CAD build for the part. Positions are in the model's coordinates, mm. Coordinates: 2 decimals unless noted, no trailing zeros. Loops run counter-clockwise (first coordinate to the right, second up) from the corner with the lowest first, then second, coordinate; pieces in that order, holes last. Notation, with made-up numbers: (25.5, 2) -> (42.5, 2) arc R20 cw to (42.5, 41) -> close; hole circle Ø3 at (19.25, 33.25). An arc over 180 degrees is marked (long way). Write each question's results on one line, items separated by ' | '.
from build123d import *

# Parameters (mm, degrees)
SKETCH_1_W             = 830
SKETCH_1_H             = 2008
SKETCH_1_W_2           = 620
SKETCH_1_H_2           = 850
EXTRUDE_1_DEPTH        = 2
SKETCH_2_W             = 810
SKETCH_2_H             = 30
CUT_EXTRUDE_1_DEPTH    = 2
SKETCH_3_W             = 2
SKETCH_3_H             = 2008
EXTRUDE_2_DEPTH        = 25.5
SKETCH_4_W             = 200
SKETCH_4_H             = 150
CUT_EXTRUDE_2_DEPTH    = 2173.927575875
SKETCH_5_W             = 30
SKETCH_5_H             = 2
SKETCH_5_W_2           = 596
SKETCH_5_W_3           = 826
EXTRUDE_3_DEPTH        = 25.5
EXTRUDE_4_DEPTH        = 5
SKETCH_8_W             = 3
SKETCH_8_H             = 8
CUT_EXTRUDE_3_DEPTH    = 813
PATTERN_LINEAR_1_COUNT = 2
PATTERN_LINEAR_1_PITCH = 1050
SKETCH_9_R             = 2.75
CUT_EXTRUDE_4_DEPTH    = 126
SKETCH_10_R            = 2.75
CUT_EXTRUDE_5_DEPTH    = 1163


with BuildPart() as part:
    # 草图1 → 凸台-拉伸1 (new body)
    with BuildSketch(Plane.XY):
        with Locations((415, -1004)):
            Rectangle(SKETCH_1_W, SKETCH_1_H)
        with Locations((415, -1133)):
            Rectangle(SKETCH_1_W_2, SKETCH_1_H_2, mode=Mode.SUBTRACT)
    extrude(amount=EXTRUDE_1_DEPTH)

    # 草图2 → 切除-拉伸1 (cut)
    with BuildSketch(Plane.XY.offset(2)):
        with Locations((415, -1658)):
            Rectangle(SKETCH_2_W, SKETCH_2_H)
        with Locations((415, -608)):
            Rectangle(SKETCH_2_W, SKETCH_2_H)
    extrude(amount=-CUT_EXTRUDE_1_DEPTH, mode=Mode.SUBTRACT)

    # 草图3 → 凸台-拉伸2 (add)
    with BuildSketch(Plane.XY):
        with Locations((1, -1004)):
            Rectangle(SKETCH_3_W, SKETCH_3_H)
        with Locations((829, -1004)):
            Rectangle(SKETCH_3_W, SKETCH_3_H)
    extrude(amount=-EXTRUDE_2_DEPTH)

    # 草图4 → 切除-拉伸2 (cut, through all)
    with BuildSketch(Plane(origin=(0, 0, 0), x_dir=(-1, 0, 0), z_dir=(0, 0, -1))):
        with Locations((-698, -1933)):
            Rectangle(SKETCH_4_W, SKETCH_4_H)
    extrude(amount=-CUT_EXTRUDE_2_DEPTH, mode=Mode.SUBTRACT)

    # 草图5 → 凸台-拉伸3 (add)
    with BuildSketch(Plane(origin=(0, 0, 0), x_dir=(-1, 0, 0), z_dir=(0, 0, -1))):
        with Locations((-813, -2007)):
            Rectangle(SKETCH_5_W, SKETCH_5_H)
        with Locations((-300, -2007)):
            Rectangle(SKETCH_5_W_2, SKETCH_5_H)
        with Locations((-415, -1)):
            Rectangle(SKETCH_5_W_3, SKETCH_5_H)
    extrude(amount=EXTRUDE_3_DEPTH)

    # 草图7 → 凸台-拉伸4 (add)
    with BuildSketch(Plane.XY.offset(2)):
        Polygon((820, -564.997302091), (820, -580), (7, -580), (7, -636), (820, -636), (820, -651), (0, -651), (0, -564.997302091), align=None)
    extrude_4 = extrude(amount=EXTRUDE_4_DEPTH)

    # 草图8 → 切除-拉伸3 (cut)
    with BuildSketch(Plane(origin=(820, 0, 0), x_dir=(0, 0, -1), z_dir=(1, 0, 0))):
        with Locations((-3.5, -576)):
            Rectangle(SKETCH_8_W, SKETCH_8_H)
        with Locations((-3.5, -640)):
            Rectangle(SKETCH_8_W, SKETCH_8_H)
    cut_extrude_3 = extrude(amount=-CUT_EXTRUDE_3_DEPTH, mode=Mode.SUBTRACT)

    # 阵列(线性)1: 凸台-拉伸4, 切除-拉伸3 ×2
    with Locations(*[(0, -i * PATTERN_LINEAR_1_PITCH, 0) for i in range(1, PATTERN_LINEAR_1_COUNT)]):
        add(extrude_4)
        add(cut_extrude_3, mode=Mode.SUBTRACT)

    # 草图9 → 切除-拉伸4 (cut)
    with BuildSketch(Plane(origin=(0, 0, 0), x_dir=(-1, 0, 0), z_dir=(0, 0, -1))):
        with Locations((-565, -695.5)):
            Circle(SKETCH_9_R)
        with Locations((-265, -695.5)):
            Circle(SKETCH_9_R)
        with Locations((-737.5, -933)):
            Circle(SKETCH_9_R)
        with Locations((-737.5, -1333)):
            Circle(SKETCH_9_R)
        with Locations((-565, -1570.5)):
            Circle(SKETCH_9_R)
        with Locations((-265, -1570.5)):
            Circle(SKETCH_9_R)
        with Locations((-92.5, -1333)):
            Circle(SKETCH_9_R)
        with Locations((-92.5, -933)):
            Circle(SKETCH_9_R)
    extrude(amount=-CUT_EXTRUDE_4_DEPTH, mode=Mode.SUBTRACT)

    # 草图10 → 切除-拉伸5 (cut)
    with BuildSketch(Plane.ZY):
        with Locations(Location((-16.5, -1978, 0), (0, 0, 270))):
            Circle(SKETCH_10_R)
        with Locations(Location((-16.5, -1158, 0), (0, 0, 270))):
            Circle(SKETCH_10_R)
        with Locations(Location((-16.5, -338, 0), (0, 0, 270))):
            Circle(SKETCH_10_R)
    extrude(amount=-CUT_EXTRUDE_5_DEPTH, mode=Mode.SUBTRACT)


solid = part.part
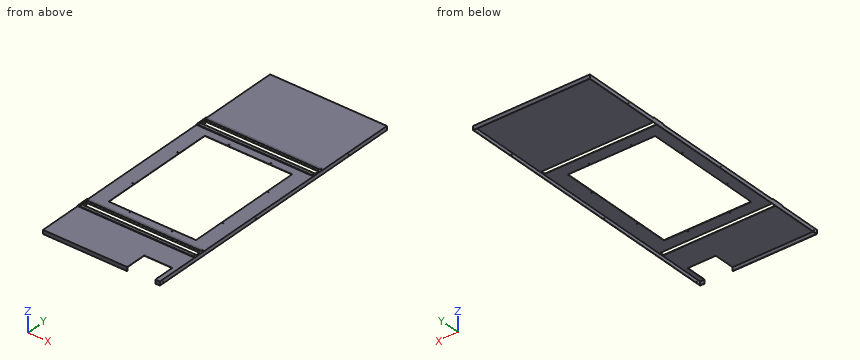
1) Slice it at B-B (x = 534). Count the separate pieces of the cut face and the enclosed holes in it, then the cut area to 3 significant figures.
Outcome:
separate pieces: 4 | enclosed holes: 0 | area: 2,500 mm^2
2) Drill centre lines: L1, parallel to X at y = -1570.5, z = 1.35; L2, parallel to Y at x = 737.5, z = 1.3; L3, parallel to X at y = -1333, z = 1. Where is each one in solid material? Low to high. Write a range as from..to.
Outcome:
L1: x = 0..262.25, 267.75..562.25, 567.75..830 | L2: y = -1858..-1673, -1643..-1335.75, -1330.25..-935.75, -930.25..-623, -593..0 | L3: x = 0..89.75, 95.25..105, 725..734.75, 740.25..830
3) Slice it at C-C (z = -6). Write the cut outline in (x, y), then the cut area to 3 significant figures.
Outcome:
outline: (0, -2008) -> (598, -2008) -> (598, -2006) -> (2, -2006) -> (2, -2) -> (828, -2) -> (828, -2006) -> (798, -2006) -> (798, -2008) -> (830, -2008) -> (830, 0) -> (0, 0) -> close | area: 10,900 mm^2
4) Slice it at D-D (y = -1083.5). Write the cut outline in (x, z).
Outcome:
outline: (0, -25.5) -> (2, -25.5) -> (2, 0) -> (105, 0) -> (105, 2) -> (0, 2) -> close; (725, 0) -> (828, 0) -> (828, -25.5) -> (830, -25.5) -> (830, 2) -> (725, 2) -> close
5) Slice it at A-A (y = -1878). Write the cut outline in (x, z), then the cut area to 3 significant figures.
Outcome:
outline: (0, -25.5) -> (2, -25.5) -> (2, 0) -> (598, 0) -> (598, 2) -> (0, 2) -> close; (798, 0) -> (828, 0) -> (828, -25.5) -> (830, -25.5) -> (830, 2) -> (798, 2) -> close | area: 1,360 mm^2
6) Pin check, flat tips, straight feed: pin 1 (3 mm diameter, centred on x = 537, z = -8.5, fed in from +Y); pin 2 (2.5 mm diameter, centred on x = 252.5, y = -1689, fed in from -Z); pin 3 (4 mm diameter, centred on y = -1623.5, z = 5, fed in from +X); pin 4 (1 mm diameter, centred on x = 364.5, y = -1743, fed in from +Z). Stop position of each tip, or through.
Outcome:
pin 1: stops at y = 0 | pin 2: stops at z = 0 | pin 3: stops at x = 820 | pin 4: stops at z = 2
